Geometry: final body of the model. Coordinates: model frame, mm. A direction names the side the tool comes from. Give positions to 0.01 mm unless a question says otherwise; leave off trailing zeros. Write each loop counter-clockwise with the first axis right and the second up, starting at its lowest first coordinate (ties: lowest second). Pieces come first, ordered by that corner, then holes. Notation, with made-up numbers: (32, 86) -> (58, 86) arc R24 ccw to (58, 102) -> close; hole circle Ø1 at (79, -29). An arc over 180 degrees is marked (long way). Answer in a Markdown table with one row per item. Add a question column.
Item 1: Section query B-B on z = 180. Output: boundary loops of the cut face in (x, y), plus the area to 3 significant figures.
Item 2: First-contact query: P1, Ø3, axis at x = -28, z = 158, coming from the -Y side; P2, Ø6.5, axis at x = -26.5, z = 42, coming from the +Y side; P3, Ø1.5, axis at x = 13.5, y = -19, coming from the +Z side. Flat tips, straight axial feed; report the tip coordinate or a pass-through.
Item 3: Access query for faces 1 (the cylindrical face through (27.349, 15.521, 184.957)), 2 (the flat face through (29, 14, 177.8)), 3 (the cylindrical face through (31.19, 18.52, 10.5)), 4 (the flat face through (-37, 0, 93)). Directions: +Z, -Z, +X, -X, +Y, -Y. A direction counts if a zero-diameter tool reaches every point of the face in a straight line with its end or side. Return the directions, or none.
Item 4: Section query C-C on x = 0. Output: boundary loops of the cut face in (y, z).
Item 5: Draft query along Y for faces 5 (the cylindrical face through (6.984, -18.521, 19.824)), 6 (the cylindrical face through (39, -18, 78)), 7 (the flat face through (37, 0, 93)). Return one class per face: +Y half, -Y half, draft (parallel to the pull), parting line (faces both ways), or undercut.
Item 6: Material intervals for probe 1 along X at (y, z) = (12, 135); probe 2 along Y at (x, z) = (-31, 62.5); probe 3 along Z at (x, y) = (25, 18), sorted ascending. Write a range as from..to.
Item 7: Section query D-D on z = 67. State how many separate pieces and enclosed holes the cut face has, plus the area to 3 significant figures.
Item 8: Section query A-A on y = -7. Output: boundary loops of the cut face in (x, z), plus the area to 3 significant figures.
```python
from build123d import *

# Parameters (mm, degrees)
EXTRUDE_1_DEPTH              = 190
SKETCH_6_R                   = 23.25
CUT_EXTRUDE_1_DEPTH          = 3
HOLE_WIZARD_6_5_6_5_1_D      = 6.5
HOLE_WIZARD_12_0_12_1_REACH  = 200.242
HOLE_WIZARD_12_0_12_1_BORE_R = 6
HOLE_WIZARD_M4_1_REACH       = 200.242
HOLE_WIZARD_M4_1_BORE_R      = 1.65
CUT_EXTRUDE_2_DEPTH          = 208.123151772
SKETCH_12_R                  = 5
EXTRUDE_2_DEPTH              = 3
HOLE_WIZARD_M5_1_D           = 4.2
HOLE_WIZARD_M3_1_D           = 2.5
HOLE_WIZARD_M3_1_DEPTH       = 3
CUT_EXTRUDE_3_REACH          = 200.242
SKETCH_17_R                  = 4


with BuildPart() as part:
    # 草图1 → 凸台-拉伸1 (new body)
    with BuildSketch(Plane.XY):
        with BuildLine():
            Line((-35, 20), (35, 20))
            ThreePointArc((35, 20), (38.535533906, 18.535533906), (40, 15))
            Line((40, 15), (40, -15))
            ThreePointArc((40, -15), (38.535533906, -18.535533906), (35, -20))
            Line((35, -20), (-35, -20))
            ThreePointArc((-35, -20), (-38.535533906, -18.535533906), (-40, -15))
            Line((-40, -15), (-40, 15))
            ThreePointArc((-40, 15), (-38.535533906, 18.535533906), (-35, 20))
        make_face()
        with BuildLine():
            Line((-37, 15), (-37, -15))
            ThreePointArc((-37, -15), (-36.414213562, -16.414213562), (-35, -17))
            Line((-35, -17), (35, -17))
            ThreePointArc((35, -17), (36.414213562, -16.414213562), (37, -15))
            Line((37, -15), (37, 15))
            ThreePointArc((37, 15), (36.414213562, 16.414213562), (35, 17))
            Line((35, 17), (-35, 17))
            ThreePointArc((-35, 17), (-36.414213562, 16.414213562), (-37, 15))
        make_face(mode=Mode.SUBTRACT)
    extrude(amount=EXTRUDE_1_DEPTH)

    # 草图6 → 切除-拉伸1 (cut)
    with BuildSketch(Plane.XZ.offset(20)):
        with Locations(Location((0, 42, 0), (0, 0, 270))):
            Circle(SKETCH_6_R)
    extrude(amount=-CUT_EXTRUDE_1_DEPTH, mode=Mode.SUBTRACT)

    # Ø6.5 (6.5) 直径孔1 (through all)
    with Locations(Plane(origin=(0, 20, 0), x_dir=(1, 0, 0), z_dir=(0, 1, 0))):
        with Locations((-25, -17), (25, -17), (25, -67), (-25, -67)):
            Hole(HOLE_WIZARD_6_5_6_5_1_D / 2)

    # Ø12.0 (12) 直径孔1 bore → Ø12.0 (12) 直径孔1 (cut, up to next)
    with BuildSketch(Plane(origin=(0, 20, 0), x_dir=(1, 0, 0), z_dir=(0, 1, 0)), mode=Mode.PRIVATE) as hole_wizard_12_0_12_1_sk1:
        with Locations((-25, -17)):
            Circle(HOLE_WIZARD_12_0_12_1_BORE_R)
    hole_wizard_12_0_12_1_tool1 = extrude(hole_wizard_12_0_12_1_sk1.sketch, amount=-HOLE_WIZARD_12_0_12_1_REACH, mode=Mode.PRIVATE) & part.part
    # Ø12.0 (12) 直径孔1 bore → Ø12.0 (12) 直径孔1 (cut, up to next)
    with BuildSketch(Plane(origin=(0, 20, 0), x_dir=(1, 0, 0), z_dir=(0, 1, 0)), mode=Mode.PRIVATE) as hole_wizard_12_0_12_1_sk2:
        with Locations((25, -17)):
            Circle(HOLE_WIZARD_12_0_12_1_BORE_R)
    hole_wizard_12_0_12_1_tool2 = extrude(hole_wizard_12_0_12_1_sk2.sketch, amount=-HOLE_WIZARD_12_0_12_1_REACH, mode=Mode.PRIVATE) & part.part
    # Ø12.0 (12) 直径孔1 bore → Ø12.0 (12) 直径孔1 (cut, up to next)
    with BuildSketch(Plane(origin=(0, 20, 0), x_dir=(1, 0, 0), z_dir=(0, 1, 0)), mode=Mode.PRIVATE) as hole_wizard_12_0_12_1_sk3:
        with Locations((25, -67)):
            Circle(HOLE_WIZARD_12_0_12_1_BORE_R)
    hole_wizard_12_0_12_1_tool3 = extrude(hole_wizard_12_0_12_1_sk3.sketch, amount=-HOLE_WIZARD_12_0_12_1_REACH, mode=Mode.PRIVATE) & part.part
    # Ø12.0 (12) 直径孔1 bore → Ø12.0 (12) 直径孔1 (cut, up to next)
    with BuildSketch(Plane(origin=(0, 20, 0), x_dir=(1, 0, 0), z_dir=(0, 1, 0)), mode=Mode.PRIVATE) as hole_wizard_12_0_12_1_sk4:
        with Locations((-25, -67)):
            Circle(HOLE_WIZARD_12_0_12_1_BORE_R)
    hole_wizard_12_0_12_1_tool4 = extrude(hole_wizard_12_0_12_1_sk4.sketch, amount=-HOLE_WIZARD_12_0_12_1_REACH, mode=Mode.PRIVATE) & part.part
    add(hole_wizard_12_0_12_1_tool1.solids().sort_by_distance((-25, 20, 17))[0], mode=Mode.SUBTRACT)
    add(hole_wizard_12_0_12_1_tool2.solids().sort_by_distance((25, 20, 17))[0], mode=Mode.SUBTRACT)
    add(hole_wizard_12_0_12_1_tool3.solids().sort_by_distance((25, 20, 67))[0], mode=Mode.SUBTRACT)
    add(hole_wizard_12_0_12_1_tool4.solids().sort_by_distance((-25, 20, 67))[0], mode=Mode.SUBTRACT)

    # M4 螺纹孔1 bore → M4 螺纹孔1 (cut, up to next)
    with BuildSketch(Plane(origin=(0, 20, 0), x_dir=(1, 0, 0), z_dir=(0, 1, 0)), mode=Mode.PRIVATE) as hole_wizard_m4_1_sk1:
        with Locations((-32.5, -9.5)):
            Circle(HOLE_WIZARD_M4_1_BORE_R)
    hole_wizard_m4_1_tool1 = extrude(hole_wizard_m4_1_sk1.sketch, amount=-HOLE_WIZARD_M4_1_REACH, mode=Mode.PRIVATE) & part.part
    # M4 螺纹孔1 bore → M4 螺纹孔1 (cut, up to next)
    with BuildSketch(Plane(origin=(0, 20, 0), x_dir=(1, 0, 0), z_dir=(0, 1, 0)), mode=Mode.PRIVATE) as hole_wizard_m4_1_sk2:
        with Locations((32.5, -9.5)):
            Circle(HOLE_WIZARD_M4_1_BORE_R)
    hole_wizard_m4_1_tool2 = extrude(hole_wizard_m4_1_sk2.sketch, amount=-HOLE_WIZARD_M4_1_REACH, mode=Mode.PRIVATE) & part.part
    # M4 螺纹孔1 bore → M4 螺纹孔1 (cut, up to next)
    with BuildSketch(Plane(origin=(0, 20, 0), x_dir=(1, 0, 0), z_dir=(0, 1, 0)), mode=Mode.PRIVATE) as hole_wizard_m4_1_sk3:
        with Locations((32.5, -74.5)):
            Circle(HOLE_WIZARD_M4_1_BORE_R)
    hole_wizard_m4_1_tool3 = extrude(hole_wizard_m4_1_sk3.sketch, amount=-HOLE_WIZARD_M4_1_REACH, mode=Mode.PRIVATE) & part.part
    # M4 螺纹孔1 bore → M4 螺纹孔1 (cut, up to next)
    with BuildSketch(Plane(origin=(0, 20, 0), x_dir=(1, 0, 0), z_dir=(0, 1, 0)), mode=Mode.PRIVATE) as hole_wizard_m4_1_sk4:
        with Locations((-32.5, -74.5)):
            Circle(HOLE_WIZARD_M4_1_BORE_R)
    hole_wizard_m4_1_tool4 = extrude(hole_wizard_m4_1_sk4.sketch, amount=-HOLE_WIZARD_M4_1_REACH, mode=Mode.PRIVATE) & part.part
    add(hole_wizard_m4_1_tool1.solids().sort_by_distance((-32.5, 20, 9.5))[0], mode=Mode.SUBTRACT)
    add(hole_wizard_m4_1_tool2.solids().sort_by_distance((32.5, 20, 9.5))[0], mode=Mode.SUBTRACT)
    add(hole_wizard_m4_1_tool3.solids().sort_by_distance((32.5, 20, 74.5))[0], mode=Mode.SUBTRACT)
    add(hole_wizard_m4_1_tool4.solids().sort_by_distance((-32.5, 20, 74.5))[0], mode=Mode.SUBTRACT)

    # 草图9 → 切除-拉伸2 (cut, through all)
    with BuildSketch(Plane(origin=(40, 0, 0), x_dir=(0, 0, -1), z_dir=(1, 0, 0))):
        Polygon((-190, 17), (-190, -20), (-156, -20), (-156, -17), align=None)
    extrude(amount=-CUT_EXTRUDE_2_DEPTH, mode=Mode.SUBTRACT)

    # 草图12 → 凸台-拉伸2 (add)
    with BuildSketch(Plane.XZ.offset(-17)):
        with Locations((-28, 160)):
            Circle(SKETCH_12_R)
        with Locations((-28, 180)):
            Circle(SKETCH_12_R)
        with Locations((28, 160)):
            Circle(SKETCH_12_R)
        with Locations((28, 180)):
            Circle(SKETCH_12_R)
    extrude(amount=EXTRUDE_2_DEPTH)

    # M5 螺纹孔1 (through all)
    with Locations(Plane(origin=(0, 20, 0), x_dir=(1, 0, 0), z_dir=(0, 1, 0))):
        with Locations((-28, -160), (-28, -180), (28, -160), (28, -180)):
            Hole(HOLE_WIZARD_M5_1_D / 2)

    # M3 螺纹孔1
    with Locations(Plane(origin=(0, -20, 0), x_dir=(-1, 0, 0), z_dir=(0, -1, 0))):
        with Locations((26.5, -42), (-26.5, -42)):
            Hole(HOLE_WIZARD_M3_1_D / 2, depth=HOLE_WIZARD_M3_1_DEPTH)

    # 草图17 → 切除-拉伸3 (cut, up to next)
    with BuildSketch(Plane(origin=(0, 20, 0), x_dir=(1, 0, 0), z_dir=(0, 1, 0)), mode=Mode.PRIVATE) as cut_extrude_3_sk1:
        with Locations(Location((-26.5, -42, 0), (0, 0, 270))):
            Circle(SKETCH_17_R)
    cut_extrude_3_tool1 = extrude(cut_extrude_3_sk1.sketch, amount=-CUT_EXTRUDE_3_REACH, mode=Mode.PRIVATE) & part.part
    # 草图17 → 切除-拉伸3 (cut, up to next)
    with BuildSketch(Plane(origin=(0, 20, 0), x_dir=(1, 0, 0), z_dir=(0, 1, 0)), mode=Mode.PRIVATE) as cut_extrude_3_sk2:
        with Locations(Location((26.5, -42, 0), (0, 0, 270))):
            Circle(SKETCH_17_R)
    cut_extrude_3_tool2 = extrude(cut_extrude_3_sk2.sketch, amount=-CUT_EXTRUDE_3_REACH, mode=Mode.PRIVATE) & part.part
    add(cut_extrude_3_tool1.solids().sort_by_distance((-26.5, 20, 42))[0], mode=Mode.SUBTRACT)
    add(cut_extrude_3_tool2.solids().sort_by_distance((26.5, 20, 42))[0], mode=Mode.SUBTRACT)


solid = part.part
```
Findings below:
| question | item | result |
|---|---|---|
| 1 | outline | (-40, 7) -> (-37, 7) -> (-37, 15) arc R2 cw to (-35, 17) -> (-33, 17) -> (-33, 14) -> (-30.1, 14) -> (-30.1, 20) -> (-35, 20) arc R5 ccw to (-40, 15) -> close; (-25.9, 14) -> (-23, 14) -> (-23, 17) -> (23, 17) -> (23, 14) -> (25.9, 14) -> (25.9, 20) -> (-25.9, 20) -> close; (30.1, 14) -> (33, 14) -> (33, 17) -> (35, 17) arc R2 cw to (37, 15) -> (37, 7) -> (40, 7) -> (40, 15) arc R5 ccw to (35, 20) -> (30.1, 20) -> close |
| 1 | area | 301 mm^2 |
| 2 | P1 | stops at y = 14 |
| 2 | P2 | stops at y = -17 |
| 2 | P3 | stops at z = 156 |
| 3 | face 1 | -Y |
| 3 | face 2 | +Z, -Z, -Y |
| 3 | face 3 | +Y |
| 3 | face 4 | +Z, -Z |
| 4 | outline | (-20, 0) -> (-17, 0) -> (-17, 18.75) -> (-20, 18.75) -> close; (-20, 65.25) -> (-17, 65.25) -> (-17, 156) -> (-20, 156) -> close; (17, 0) -> (20, 0) -> (20, 190) -> (17, 190) -> close |
| 5 | face 5 | draft |
| 5 | face 6 | -Y half |
| 5 | face 7 | undercut |
| 6 | probe 1 | x = -40..-37, 37..40 |
| 6 | probe 2 | y = -20..-17, 17..20 |
| 6 | probe 3 | z = 0..11, 23..38.29, 45.71..61, 73..190 |
| 7 | separate pieces | 4 |
| 7 | enclosed holes | 0 |
| 7 | area | 555 mm^2 |
| 8 | outline | (-40, 0) -> (-37, 0) -> (-37, 166) -> (-40, 166) -> close; (37, 0) -> (40, 0) -> (40, 166) -> (37, 166) -> close |
| 8 | area | 996 mm^2 |
